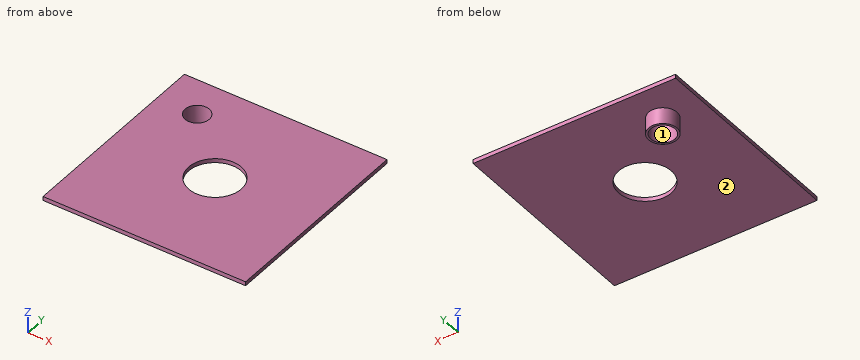
from build123d import *

# Parameters (mm, degrees)
SKETCH1_W           = 500
SKETCH1_H           = 500
SKETCH1_R           = 65
SKETCH1_R_2         = 30
BOSS_EXTRUDE1_DEPTH = 10
SKETCH2_R           = 35
SKETCH2_R_2         = 29.957117648
BOSS_EXTRUDE2_DEPTH = 50


with BuildPart() as part:
    # Sketch1 → Boss-Extrude1 (new body)
    with BuildSketch(Plane.XY):
        with Locations((250, 250)):
            Rectangle(SKETCH1_W, SKETCH1_H)
        with Locations((250, 250)):
            Circle(SKETCH1_R, mode=Mode.SUBTRACT)
        with Locations((97.913524384, 404.851684263)):
            Circle(SKETCH1_R_2, mode=Mode.SUBTRACT)
    extrude(amount=BOSS_EXTRUDE1_DEPTH)

    # Sketch2 → Boss-Extrude2 (add)
    with BuildSketch(Plane.XY.offset(10)):
        with Locations((97.913524384, 404.851684263)):
            Circle(SKETCH2_R)
        with Locations((97.913524384, 404.851684263)):
            Circle(SKETCH2_R_2, mode=Mode.SUBTRACT)
    extrude(amount=-BOSS_EXTRUDE2_DEPTH)


solid = part.part
Input: part model. Units: mm. Frame: model coordinates. Face numbers are marked on the shaded views. Give positions to 0.01 mm unless a question says otherwise; leave off trailing zeros. Order: outer loops, then holes, each group sorted by start corner. A loop starts at its lowest first (then second) coordinate and runs counter-clockwise, first axis right, second up. Notation, with made-up numbers: (68, 61.25) - (118, 61.25) arc R19 ccw to (118, 78.25) - close; hole circle Ø2 at (78, 82). An arc over 180 degrees is marked (long way). Write each question's results on one line, items separated by ' | '.
Item 1: Draft query along X for the marked faces 1 and 2. Return one class per face: released by +X, released by -X, zero draft, split by the parting line, or undercut.
A:
face 1: undercut | face 2: zero draft
Item 2: Material intervals for line 1 along Y through (x, z) = (250, 6.25); line 2 along Z through (x, y) = (392, 102); line 3 along Y through (x, z) = (125.5, -10.5), sorted ascending.
A:
line 1: y = 0 to 185, 315 to 500 | line 2: z = 0 to 10 | line 3: y = 383.31 to 393.17, 416.53 to 426.39
Item 3: Contact query for flat-ended pins moving along their axis: pin 1 Ø10 at (x, z) = (319, -6.5) entering from +Y; pin 2 Ø8 at (x, z) = (129, -10.5) entering from +Y; pin 3 Ø8 at (x, z) = (61, -3) entering from +Y. Output: stop coordinate, or through.
A:
pin 1: passes through | pin 2: stops at y = 427.02 | pin 3: stops at y = 500
Item 4: Section D-D (z = -25.5). Return loops of the section in (x, y).
A:
outline: circle Ø70 at (97.91, 404.85); hole circle Ø59.91 at (97.91, 404.85)
Item 5: Section A-A (y = 250). Return loops of the section in (x, z).
A:
outline: (0, 0) - (185, 0) - (185, 10) - (0, 10) - close; (315, 0) - (500, 0) - (500, 10) - (315, 10) - close
Item 6: Section C-C (x = 454.5). Return loops of the section in (y, z).
A:
outline: (0, 0) - (500, 0) - (500, 10) - (0, 10) - close
